from build123d import *

# Parameters (mm, degrees)
SKETCH_1_R      = 7
SKETCH_1_R_2    = 5.1
EXTRUDE_1_DEPTH = 29.15
CHAMFER_1_SIZE  = 0.3
CHAMFER_2_SIZE  = 0.3


with BuildPart() as part:
    # 草图1 → 凸台-拉伸1 (new body)
    with BuildSketch(Plane.XY):
        Circle(SKETCH_1_R)
        Circle(SKETCH_1_R_2, mode=Mode.SUBTRACT)
    extrude(amount=EXTRUDE_1_DEPTH)

    # 倒角1
    chamfer_1_edges = [part.edges().sort_by_distance(p)[0] for p in [
        (-7, 0, 0),
    ]]
    chamfer(chamfer_1_edges, length=CHAMFER_1_SIZE)

    # 倒角2
    chamfer_2_edges = [part.edges().sort_by_distance(p)[0] for p in [
        (-7, 0, 29.15),
        (-5.1, 0, 0),
        (-5.1, 0, 29.15),
    ]]
    chamfer(chamfer_2_edges, length=CHAMFER_2_SIZE)


solid = part.part
Verification items for the finished model (mm, model axes). Coordinates: 2 decimals unless noted, no trailing zeros. Order: outer loops, then holes, each group sorted by start corner. A loop starts at its lowest first (then second) coordinate and runs counter-clockwise, first axis right, second up. Notation, with made-up numbers: M 72.25,-10.5 L 88.25,-10.5 A28 ccw 88.25,27.5 Z; hole C -7,48.5 d5. An arc over 180 degrees is marked long. Return JSON: item names as keys, results as strings.
1) Release check for a two-part mould opening along X. For faces 1 (the cylindrical face through (6.466, -2.681, 14.375)), 2 (the cylindrical face through (2.4, -4.5, 14.4)) record: +X half, -X half, draft (parallel to the pull), parting line (faces both ways), or undercut.
Answer list:
{"face 1": "parting line", "face 2": "undercut"}
2) Cross-section at C-C, the plane z = 3.5. Record the boundary of the cut face in (x, y).
Answer list:
{"outline": "C 0,0 d14; hole C 0,0 d10.2"}
3) Thickness scan on L1, parallel to Y at x = 0, z = 6.5; L2, parallel to X at y = 1.25, z = 24.25; L3, parallel to Y at x = -4.5, z = 27.75. Record the ranges inside material, lowest first. Write a range as [from, to].
Answer list:
{"L1": "[-7, -5.1], [5.1, 7]", "L2": "[-6.89, -4.94], [4.94, 6.89]", "L3": "[-5.36, -2.4], [2.4, 5.36]"}
4) Gauge pin test, flat ends, axial feed: pin 1 (1 mm diameter, centred on x = 0.5, z = 12.5, fed in from -Y); pin 2 (4 mm diameter, centred on x = -3, z = 10, fed in from +Y); pin 3 (3 mm diameter, centred on y = -2.5, z = 8.5, fed in from +X); pin 4 (2 mm diameter, centred on y = -3, z = 10, fed in from +X). Record the tip position at first contact, or that the pin passes through.
Answer list:
{"pin 1": "y = -7", "pin 2": "y = 6.93", "pin 3": "x = 6.93", "pin 4": "x = 6.71"}
5) Cross-section at A-A, the plane x = 0. Record the boundary of the cut face in (y, z).
Answer list:
{"outline": "M -7,0.3 L -6.7,0 L -5.4,0 L -5.1,0.3 L -5.1,28.85 L -5.4,29.15 L -6.7,29.15 L -7,28.85 Z; M 5.1,0.3 L 5.4,0 L 6.7,0 L 7,0.3 L 7,28.85 L 6.7,29.15 L 5.4,29.15 L 5.1,28.85 Z"}
